Verification items for the finished model (mm, model axes). Face numbers are marked on the shaded views. A direction names the side the tool comes from. Give positions to 0.01 mm unless a question says otherwise; leave off trailing zeros. Loops run counter-clockwise (first coordinate to the right, second up) from the corner with the lowest first, then second, coordinate; pieces in that order, holes last. Notation, with made-up numbers: (56, -21.75) - (107, -21.75) arc R31 cw to (107, 4.25) - close; hole circle Ø1 at (-2.75, 43.25). An arc over 180 degrees is marked (long way). Put each result on its own line as item: value. Start each with the question number.
```python
from build123d import *

# Parameters (mm, degrees)
SKETCH1_R           = 25
SKETCH1_R_2         = 16
BOSS_EXTRUDE1_DEPTH = 3
SKETCH2_W           = 52
SKETCH2_H           = 52
SKETCH2_R           = 16
BOSS_EXTRUDE2_DEPTH = 8
SKETCH3_R           = 2
CUT_EXTRUDE1_DEPTH  = 39.495320082
SKETCH4_R           = 2
CUT_EXTRUDE2_DEPTH  = 38.747710768
SKETCH5_R           = 3.5
CUT_EXTRUDE3_DEPTH  = 3


with BuildPart() as part:
    # Sketch1 → Boss-Extrude1 (new body)
    with BuildSketch(Plane.XY):
        Circle(SKETCH1_R)
        Circle(SKETCH1_R_2, mode=Mode.SUBTRACT)
    extrude(amount=BOSS_EXTRUDE1_DEPTH)

    # Sketch2 → Boss-Extrude2 (add)
    with BuildSketch(Plane.XY.offset(3)):
        with Locations((0.170396792, 0)):
            Rectangle(SKETCH2_W, SKETCH2_H)
        Circle(SKETCH2_R, mode=Mode.SUBTRACT)
    extrude(amount=BOSS_EXTRUDE2_DEPTH)

    # Sketch3 → Cut-Extrude1 (cut, through all)
    with BuildSketch(Plane(origin=(0, 0, 0), x_dir=(-1, 0, 0), z_dir=(0, 0, -1))):
        with Locations((0, 20.5)):
            Circle(SKETCH3_R)
        with Locations((17.753520778, 10.25)):
            Circle(SKETCH3_R)
        with Locations((17.753520778, -10.25)):
            Circle(SKETCH3_R)
        with Locations((0, -20.5)):
            Circle(SKETCH3_R)
        with Locations((-17.753520778, -10.25)):
            Circle(SKETCH3_R)
        with Locations((-17.753520778, 10.25)):
            Circle(SKETCH3_R)
    extrude(amount=-CUT_EXTRUDE1_DEPTH, mode=Mode.SUBTRACT)

    # Sketch4 → Cut-Extrude2 (cut, through all)
    with BuildSketch(Plane(origin=(0, 0, 3), x_dir=(-1, 0, 0), z_dir=(0, 0, -1))):
        with Locations((-21, 21)):
            Circle(SKETCH4_R)
        with Locations(Location((21, 21, 0), (0, 0, 180))):
            Circle(SKETCH4_R)
        with Locations((21, -21)):
            Circle(SKETCH4_R)
        with Locations(Location((-21, -21, 0), (0, 0, 180))):
            Circle(SKETCH4_R)
    extrude(amount=-CUT_EXTRUDE2_DEPTH, mode=Mode.SUBTRACT)

    # Sketch5 → Cut-Extrude3 (cut)
    with BuildSketch(Plane(origin=(0, 0, 0), x_dir=(-1, 0, 0), z_dir=(0, 0, -1))):
        with Locations((0, 20.5)):
            Circle(SKETCH5_R)
        with Locations((17.753520778, 10.25)):
            Circle(SKETCH5_R)
        with Locations((17.753520778, -10.25)):
            Circle(SKETCH5_R)
        with Locations((0, -20.5)):
            Circle(SKETCH5_R)
        with Locations((-17.753520778, -10.25)):
            Circle(SKETCH5_R)
        with Locations((-17.753520778, 10.25)):
            Circle(SKETCH5_R)
    extrude(amount=-CUT_EXTRUDE3_DEPTH, mode=Mode.SUBTRACT)


solid = part.part
```
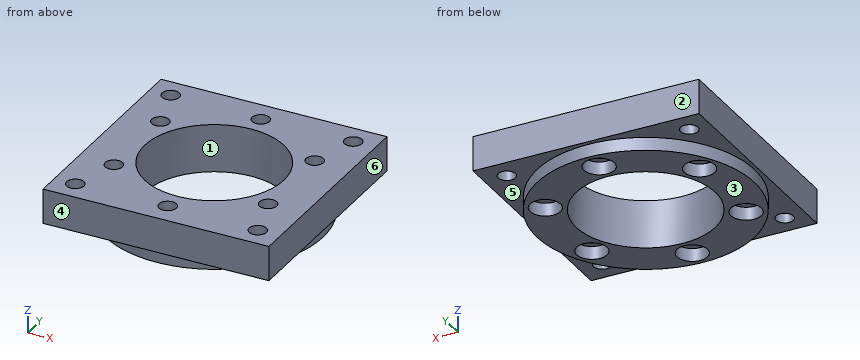
1) Section check B-B, the plane x = 0. Enter the section's corners in (y, z).
2) Section check C-C, the plane z = 2. Enter the section's corners in (x, y).
3) Section check D-D, the plane z = 4.75. State how many separate pieces and enclosed holes the cut face has, plus the area to 3 significant figures.
4) Draft check along Y on the marked faces 1, 2, 3 and 4. Enter one of: pulls with the +Y half, pulls with the -Y half, needs draft (parallel to the pull), parting line crosses it, or undercut.
5) Set-up check for the marked faces 5 and 6: record each of +Z, -Z, +X, -X, +Y, -Y from which the full face is reachable in a straight line by a thin tool's end or side.
6) Section check A-A, the plane y = 0. Enter the section's corners in (x, z).
7) Depth check by flat-ended pin: P1, Ø2, axis at x = 1, y = 22, coming from the -Z side; P2, Ø1.5, axis at x = 16.5, z = 2, coming from the -Y side. Enter the tip coordinate at first touch or a pass-through.
8) Scan lines: line 1 along Y through (x, z) = (0, 1.35); line 2 along Y through (x, z) = (0, 5.5); line 3 along X through (y, z) = (-21.5, 9.75). Record each from-to range of solid material in increasing order. Write a range as from..to.
Results are:
1. outline: (-26, 3) - (-25, 3) - (-25, 0) - (-24, 0) - (-24, 3) - (-22.5, 3) - (-22.5, 11) - (-26, 11) - close; (-18.5, 3) - (-17, 3) - (-17, 0) - (-16, 0) - (-16, 11) - (-18.5, 11) - close; (16, 0) - (17, 0) - (17, 3) - (18.5, 3) - (18.5, 11) - (16, 11) - close; (22.5, 3) - (24, 3) - (24, 0) - (25, 0) - (25, 3) - (26, 3) - (26, 11) - (22.5, 11) - close
2. outline: circle Ø50 at (0, 0); hole circle Ø7 at (-17.75, -10.25); hole circle Ø7 at (-17.75, 10.25); hole circle Ø32 at (0, 0); hole circle Ø7 at (0, -20.5); hole circle Ø7 at (0, 20.5); hole circle Ø7 at (17.75, -10.25); hole circle Ø7 at (17.75, 10.25)
3. separate pieces: 1
3. enclosed holes: 11
3. area: 1,770 mm2
4. face 1: undercut
4. face 2: pulls with the +Y half
4. face 3: needs draft
4. face 4: pulls with the -Y half
5. face 5: -Z
5. face 6: +Z, -Z, +X, +Y, -Y
6. outline: (-25.83, 3) - (-25, 3) - (-25, 0) - (-16, 0) - (-16, 11) - (-25.83, 11) - close; (16, 0) - (25, 0) - (25, 3) - (26.17, 3) - (26.17, 11) - (16, 11) - close
7. P1: stops at z = 3
7. P2: stops at y = -19.41
8. line 1: y = -25..-24, -17..-16, 16..17, 24..25
8. line 2: y = -26..-22.5, -18.5..-16, 16..18.5, 22.5..26
8. line 3: x = -25.83..-22.94, -19.06..-1.73, 1.73..19.06, 22.94..26.17
